from build123d import *

# Parameters (mm, degrees)
BASE_PLATE_SKETCH_W        = 68
BASE_PLATE_SKETCH_H        = 65
BASE_PLATE_68X65_DEPTH     = 9
UPRIGHT_BLOCK_DEPTH        = 9
SECOND_UPRIGHT_BLOCK_DEPTH = 9
SIDE_WEB_SKETCH_W          = 34
SIDE_WEB_SKETCH_H          = 14
SIDE_WEB_DEPTH             = 65
UPPER_SLOT_7X14_DEPTH      = 13
LOWER_SLOT_7X14_DEPTH      = 13
THROUGH_CHANNEL_SKETCH_W   = 14
THROUGH_CHANNEL_SKETCH_H   = 9
THROUGH_CHANNEL_DEPTH      = 65
BEARING_HUB_SKETCH_R       = 15
BEARING_HUB_DEPTH          = 37
HUB_START                  = 3
HUB_COLLAR_SKETCH_30_R     = 15
HUB_COLLAR_30_DEPTH        = 3
CENTER_BORE_SKETCH_18_R    = 9
CENTER_BORE_18_DEPTH       = 65
SIDE_POCKET_SKETCH_R       = 5
SIDE_POCKET_CUT_DEPTH      = 9


with BuildPart() as part:
    # Base Plate Sketch → Base Plate 68x65 (new body)
    with BuildSketch(Plane.XY):
        with Locations((34, 32.5)):
            Rectangle(BASE_PLATE_SKETCH_W, BASE_PLATE_SKETCH_H)
    extrude(amount=BASE_PLATE_68X65_DEPTH)

    # Upright Block Sketch → Upright Block (add)
    with BuildSketch(Plane.XZ):
        Polygon((0, 9), (68, 9), (51, 28), (51, 42), (34, 42), (17, 42), (17, 28), align=None)
    extrude(amount=-UPRIGHT_BLOCK_DEPTH)

    # Second Upright Sketch → Second Upright Block (add)
    with BuildSketch(Plane(origin=(0, 65, 0), x_dir=(1, 0, 0), z_dir=(0, 1, 0))):
        Polygon((34, -42), (51, -42), (51, -28), (68, -9), (0, -9), (17, -28), (17, -42), align=None)
    extrude(amount=-SECOND_UPRIGHT_BLOCK_DEPTH)

    # Side Web Sketch → Side Web (add)
    with BuildSketch(Plane.XZ):
        with Locations((34, 35)):
            Rectangle(SIDE_WEB_SKETCH_W, SIDE_WEB_SKETCH_H)
    extrude(amount=-SIDE_WEB_DEPTH)

    # Upper Slot Sketch → Upper Slot 7x14 (cut)
    with BuildSketch(Plane.XZ):
        Polygon((34, 42), (41, 42), (41, 0), (27, 0), (27, 42), align=None)
    extrude(amount=-UPPER_SLOT_7X14_DEPTH, mode=Mode.SUBTRACT)

    # Lower Slot Sketch → Lower Slot 7x14 (cut)
    with BuildSketch(Plane(origin=(0, 65, 0), x_dir=(1, 0, 0), z_dir=(0, 1, 0))):
        Polygon((34, -42), (41, -42), (41, 0), (27, 0), (27, -42), align=None)
    extrude(amount=-LOWER_SLOT_7X14_DEPTH, mode=Mode.SUBTRACT)

    # Through Channel Sketch → Through Channel (cut)
    with BuildSketch(Plane.XZ.offset(-13)):
        with Locations((34, 4.5)):
            Rectangle(THROUGH_CHANNEL_SKETCH_W, THROUGH_CHANNEL_SKETCH_H)
    extrude(amount=-THROUGH_CHANNEL_DEPTH, mode=Mode.SUBTRACT)

    # Bearing Hub Sketch → Bearing Hub (add)
    with BuildSketch(Plane.ZY.offset(-17)):
        with Locations((34, 32.5)):
            Circle(BEARING_HUB_SKETCH_R)
    extrude(amount=-BEARING_HUB_DEPTH)

    # Hub Collar Sketch Ø30 → Hub Collar Ø30 (add)
    with BuildSketch(Plane.ZY.offset(-17).offset(HUB_START)):
        with Locations((34, 32.5)):
            Circle(HUB_COLLAR_SKETCH_30_R)
    extrude(amount=-HUB_COLLAR_30_DEPTH)

    # Center Bore Sketch Ø18 → Center Bore Ø18 (cut)
    with BuildSketch(Plane.ZY.offset(-14)):
        with Locations((34, 32.5)):
            Circle(CENTER_BORE_SKETCH_18_R)
    extrude(amount=-CENTER_BORE_18_DEPTH, mode=Mode.SUBTRACT)

    # Side Pocket Sketch → Side Pocket Cut (cut)
    with BuildSketch(Plane(origin=(0, 0, 0), x_dir=(-1, 0, 0), z_dir=(0, 0, -1))):
        with Locations((-59, 32.5)):
            Circle(SIDE_POCKET_SKETCH_R)
        with Locations((-9, 32.5)):
            Circle(SIDE_POCKET_SKETCH_R)
    extrude(amount=-SIDE_POCKET_CUT_DEPTH, mode=Mode.SUBTRACT)


solid = part.part
Design review of the part built by this model. Coordinates are the model's own, in mm. A direction names the side the tool comes from. Coordinates: 2 decimals unless noted, no trailing zeros. Loops run counter-clockwise (first coordinate to the right, second up) from the corner with the lowest first, then second, coordinate; pieces in that order, holes last. Notation, with made-up numbers: M 54.25,-25.75 L 79.25,-25.75 A15 cw 79.25,-20.75 Z; hole C -21,51.25 d3. An arc over 180 degrees is marked long. Use one line per item in the form item = value.
(1) Clearance check with flat-ended pins moving along their axes: P1, Ø2, axis at x = 43, y = 34, coming from the +Z side; P2, Ø1.5, axis at x = 38, y = 18.5, coming from the -Z side; P3, Ø11, axis at y = 56, z = 36.5, coming from the -X side; P4, Ø1.5, axis at x = 39.5, y = 55.5, coming from the +Z side. State where each tip first meets the part, or that it passes through.
Return value:
P1 = 48.99
P2 = 26.97
P3 = 17
P4 = through
(2) Consider section B-B (y = 10). Write out the cut boundary in (x, z).
Return value:
outline = M 0,0 L 27,0 L 27,9 L 0,9 Z; M 17,28 L 27,28 L 27,42 L 17,42 Z; M 41,0 L 68,0 L 68,9 L 41,9 Z; M 41,28 L 51,28 L 51,42 L 41,42 Z
(3) For faces 1 (the face through (54, 26, 40.5)), 2 (the face through (34, 14, 42)), 3 (the face through (51, 56, 16)), list the 3-axis set-ups (+Z, -Z, +X, -X, +Y, -Y) from which the entire face can be reached by the end or side of a thin tool; tool diameter is ignored.
Return value:
face_1 = +Z, +X
face_2 = +Z, +X, -X, -Y
face_3 = +X, -X
(4) For line 1 along Z through (x, y) = (45, 32); line 2 along X through (y, z) = (6.5, 39.5); line 3 along Y through (x, z) = (44, 34), list the stretches that pass through material, from the lowest coordinate up. Write a range as from..to.
Return value:
line_1 = 0..9, 19.01..25.01, 42.99..48.99
line_2 = 17..27, 41..51
line_3 = 0..23.5, 41.5..65
(5) Consider section A-A (z = 34). Write out the cut boundary in (x, y), and give its area (3 significant figures).
Return value:
outline = M 14,17.5 L 17,17.5 L 17,0 L 27,0 L 27,13 L 41,13 L 41,0 L 51,0 L 51,17.5 L 54,17.5 L 54,23.5 L 14,23.5 Z; M 14,41.5 L 54,41.5 L 54,47.5 L 51,47.5 L 51,65 L 41,65 L 41,52 L 27,52 L 27,65 L 17,65 L 17,47.5 L 14,47.5 Z
area = 1,310 mm2
(6) Draft analysis for pull direction X (two halves, no side actions). For faces 4 (the face through (4.23, 34, 4.44)), 5 (the face through (68, 32, 4)), 6 (the face through (51, 33, 9)), 7 (the face through (34, 52, 35)), state which applies: pulls with the +X half, pulls with the -X half, needs draft (parallel to the pull), parting line crosses it, or undercut.
Return value:
face_4 = undercut
face_5 = pulls with the +X half
face_6 = needs draft
face_7 = undercut
(7) Consider section D-D (y = 32.5). Write out the cut boundary in (x, z).
Return value:
outline = M 0,0 L 4,0 L 4,9 L 0,9 Z; M 14,0 L 27,0 L 27,9 L 14,9 Z; M 14,19 L 54,19 L 54,25 L 14,25 Z; M 14,43 L 54,43 L 54,49 L 14,49 Z; M 41,0 L 54,0 L 54,9 L 41,9 Z; M 64,0 L 68,0 L 68,9 L 64,9 Z
(8) Consider section C-C (z = 6). Write out the cut boundary in (x, y).
Return value:
outline = M 0,0 L 27,0 L 27,65 L 0,65 Z; M 41,0 L 68,0 L 68,65 L 41,65 Z; hole C 9,32.5 d10; hole C 59,32.5 d10
